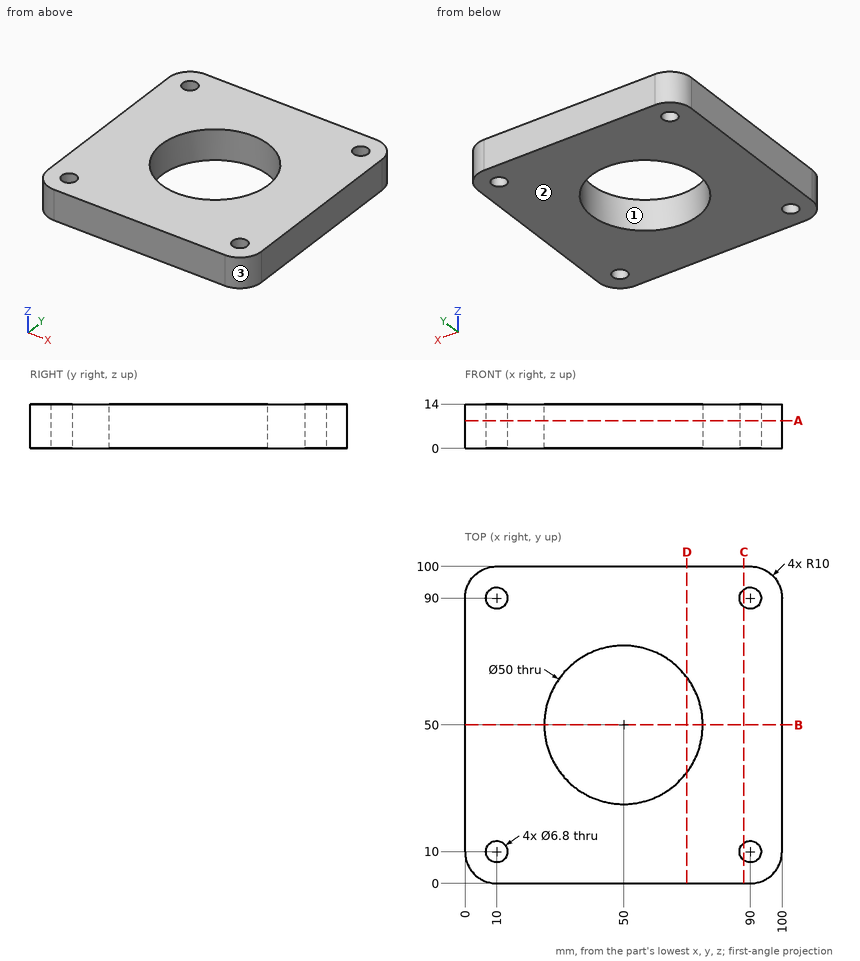
Here's the drawing with two shaded views (mm, measured from the low corner). I have some questions. Give positions to 0.01 mm unless a question says otherwise; leave off trailing zeros. Loops run counter-clockwise (first coordinate to the right, second up) from the corner with the lowest first, then second, coordinate; pieces in that order, holes last. Notation, with made-up numbers: (-35, 59.25) -> (24, 59.25) arc R23 ccw to (24, 98.25) -> close; hole circle Ø4 at (33.25, 18.25). An arc over 180 degrees is marked (long way). One line per item, written item: value.
Q1. Suppose I cut it at D-D on x = 70. Please give me the cut outline in (y, z), then the cut area to 3 significant figures.
Answers follow:
outline: (0, 0) -> (35, 0) -> (35, 14) -> (0, 14) -> close; (65, 0) -> (100, 0) -> (100, 14) -> (65, 14) -> close
area: 980 mm^2
Q2. Suppose I cut it at A-A on z = 8.75. Please give me the cut outline in (x, y).
Answers follow:
outline: (0, 10) arc R10 ccw to (10, 0) -> (90, 0) arc R10 ccw to (100, 10) -> (100, 90) arc R10 ccw to (90, 100) -> (10, 100) arc R10 ccw to (0, 90) -> close; hole circle Ø6.8 at (10, 10); hole circle Ø6.8 at (10, 90); hole circle Ø50 at (50, 50); hole circle Ø6.8 at (90, 10); hole circle Ø6.8 at (90, 90)
Q3. I'm going to push a flat-ended pin straight in: pin 1 Ø5.5 at (x, y) = (10, 10) entering from -Z. Where does the tip first touch, or does it pass through?
Answers follow:
pin 1: through
Q4. We'd pull the mould along X, two halves only. Please class the marked faces 1, 2 and 3: pulls with the +X half, pulls with the -X half, needs draft (parallel to the pull), parting line crosses it, or undercut.
Answers follow:
face 1: undercut
face 2: needs draft
face 3: pulls with the +X half
Q5. Suppose I cut it at B-B on y = 50. Please give me the cut outline in (x, z), then the cut area to 3 significant figures.
Answers follow:
outline: (0, 0) -> (25, 0) -> (25, 14) -> (0, 14) -> close; (75, 0) -> (100, 0) -> (100, 14) -> (75, 14) -> close
area: 700 mm^2
Q6. Suppose I cut it at C-C on x = 88. Please give me the cut outline in (y, z), then the cut area to 3 significant figures.
Answers follow:
outline: (0, 0) -> (7.25, 0) -> (7.25, 14) -> (0, 14) -> close; (12.75, 0) -> (87.25, 0) -> (87.25, 14) -> (12.75, 14) -> close; (92.75, 0) -> (100, 0) -> (100, 14) -> (92.75, 14) -> close
area: 1,250 mm^2
Q7. If I drill on line 1 along Y through (x, z) = (10, 7); line 2 along Y through (x, z) = (50, 7.5); line 3 along Y through (x, z) = (32, 3.75), over which ranges is the centre line in solid material (lowest first)?
Answers follow:
line 1: 0 to 6.6, 13.4 to 86.6, 93.4 to 100
line 2: 0 to 25, 75 to 100
line 3: 0 to 32.65, 67.35 to 100
